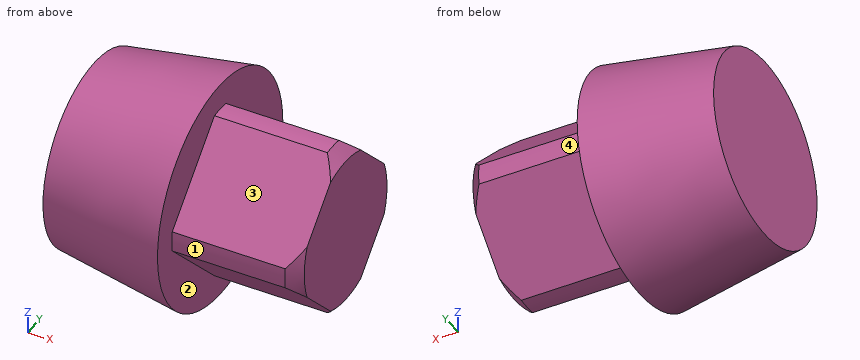
```python
from build123d import *

# Parameters (mm, degrees)
CHAMFER1_SIZE      = 2
CUT_EXTRUDE1_START = -20
CUT_EXTRUDE1_DEPTH = 20
CIRPATTERN1_COUNT  = 4


with BuildPart() as part:
    # Sketch1 → Revolve1 (revolve)
    with BuildSketch(Plane.XY, mode=Mode.PRIVATE) as revolve1_sk:
        Polygon((0, 0), (20, 0), (40, 0), (40, 14), (20, 14), (20, 18.177165354), (0, 15), align=None)
    revolve(revolve1_sk.sketch.rotate(Axis((20, 0, 0), (1, 0, 0)), 90), axis=Axis((20, 0, 0), (1, 0, 0)))

    # Chamfer1
    chamfer1_edges = [part.edges().sort_by_distance(p)[0] for p in [
        (40, 0, -14),
    ]]
    chamfer(chamfer1_edges, length=CHAMFER1_SIZE)

    # Sketch2 → Cut-Extrude1 (cut)
    with BuildSketch(Plane(origin=(40, 0, 0), x_dir=(0, 0, -1), z_dir=(1, 0, 0)).offset(CUT_EXTRUDE1_START)):
        with BuildLine():
            Line((11.169339585, 4.387009601), (13.90189895, 1.654450236))
            ThreePointArc((13.90189895, 1.654450236), (9.899494937, 9.899494937), (1.654450236, 13.90189895))
            Line((1.654450236, 13.90189895), (4.387009601, 11.169339585))
            ThreePointArc((4.387009601, 11.169339585), (8.485281374, 8.485281374), (11.169339585, 4.387009601))
        make_face()
        with BuildLine():
            Line((4.387009601, 11.169339585), (11.169339585, 4.387009601))
            ThreePointArc((11.169339585, 4.387009601), (8.485281374, 8.485281374), (4.387009601, 11.169339585))
        make_face()
    cut_extrude1 = extrude(amount=CUT_EXTRUDE1_DEPTH, mode=Mode.SUBTRACT)

    # CirPattern1: Cut-Extrude1 ×4 about axis
    cirpattern1_axis = Axis((0, 0, 0), (1, 0, 0))
    for i in range(1, CIRPATTERN1_COUNT):
        add(cut_extrude1.rotate(cirpattern1_axis, i * 360 / CIRPATTERN1_COUNT), mode=Mode.SUBTRACT)


solid = part.part
```
The model under review builds one solid part; all positions refer to its coordinate system, in mm. Face numbers are marked on the shaded views. A direction names the side the tool comes from. Give positions to 0.01 mm unless a question says otherwise; leave off trailing zeros. Write each loop counter-clockwise with the first axis right and the second up, starting at its lowest first coordinate (ties: lowest second). Pieces come first, ordered by that corner, then holes.
(1) Consider section A-A, the plane y = 0. Give the boundary of the cut face in (x, z), and give its area (3 significant figures).
(2) Consider section D-D, the plane x = 3.5. Give the boundary of the cut face in (y, z), and give its area (3 significant figures).
(3) For P1, Ø6, axis at x = 26, z = 1.5, coming from the +Y side; P2, Ø8, axis at x = 35, y = -8, coming from the +Z side; P3, Ø1.5, axis at x = 16.5, y = 6.5, coming from the +Z side, all flat-tipped, find the tip position at first contact; note any pin that passes through.
(4) Consider section C-C, the plane x = 16.5. Give the boundary of the cut face in (y, z), and give its area (3 significant figures).
(5) Tool access review of the marked faces 1, 2, 3 and 4: name each direction out of +Z, -Z, +X, -X, +Y, -Y from which nothing blocks a thin tool from reaching the whole face with its end or side.
(6) To check wall thickness, follow L1, parallel to Z at x = 31.5, y = 0; L2, parallel to X at y = 8, z = 11. State the ranges of each line that lie inside material, in increasing order.
Returned:
1. outline: (0, -15) - (20, -18.18) - (20, -14) - (38, -14) - (40, -12) - (40, 12) - (38, 14) - (20, 14) - (20, 18.18) - (0, 15) - close
1. area: 1,220 mm2
2. outline: circle Ø31.11 at (0, 0)
2. area: 760 mm2
3. P1: stops at y = 14
3. P2: stops at z = 11.56
3. P3: stops at z = 16.69
4. outline: circle Ø35.24 at (0, 0)
4. area: 975 mm2
5. face 1: +X, -Y
5. face 2: +X
5. face 3: +Z, +X, -Y
5. face 4: +X, +Y
6. L1: z = -14 to 14
6. L2: x = 0 to 20
